Could you check a few things on this drawing? It's one solid part, dimensions in mm from its lowest x, y, z. A direction names the side the tool comes from. Give positions to 0.01 mm unless a question says otherwise; leave off trailing zeros. Order: outer loops, then holes, each group sorted by start corner. A loop starts at its lowest first (then second) coordinate and runs counter-clockwise, first axis right, second up.
Item 1: If we mould it in two halves opening along X, with no side actions, what happens to the marked faces 1, 2 and 3? For each: +X half, -X half, draft (parallel to the pull), parting line (faces both ways), or undercut.
Item 2: I want a section at D-D, the plane z = 12. Write out the boundary of the cut face in (x, y), then the cut area to 3 significant figures.
Item 3: I want a section at A-A, the plane z = 7.5. Write out the boundary of the cut face in (x, y).
Item 4: I want a section at C-C, the plane x = 7.5. Write out the boundary of the cut face in (y, z).
Item 5: Which directions (+Z, -Z, +X, -X, +Y, -Y) give clear straight access to the entire face, cutting with the end or side of a thin tool? Please do the marked faces 4, 5 and 6.
Item 6: If I drill on line 1 along Z through (x, y) = (42.5, 2); line 2 along Y through (x, z) = (25, 6.5); line 3 along X through (y, z) = (20.5, 7), over which ranges is the centre line in solid material (lowest first)?
Item 7: I'm going to push flat-ended pins straight in: pin 1 Ø5.5 at (x, y) = (25, 19) entering from +Z; pin 2 Ø7.5 at (y, z) = (21, 8.5) entering from +X; pin 3 Ø7.5 at (x, z) = (4.5, 7.5) entering from +Y; pin 4 Ø7.5 at (y, z) = (18, 9.5) entering from -X. Where does each tip first touch, or does it pass through?
Item 8: I want a section at B-B, the plane y = 19. Write out the boundary of the cut face in (x, z).
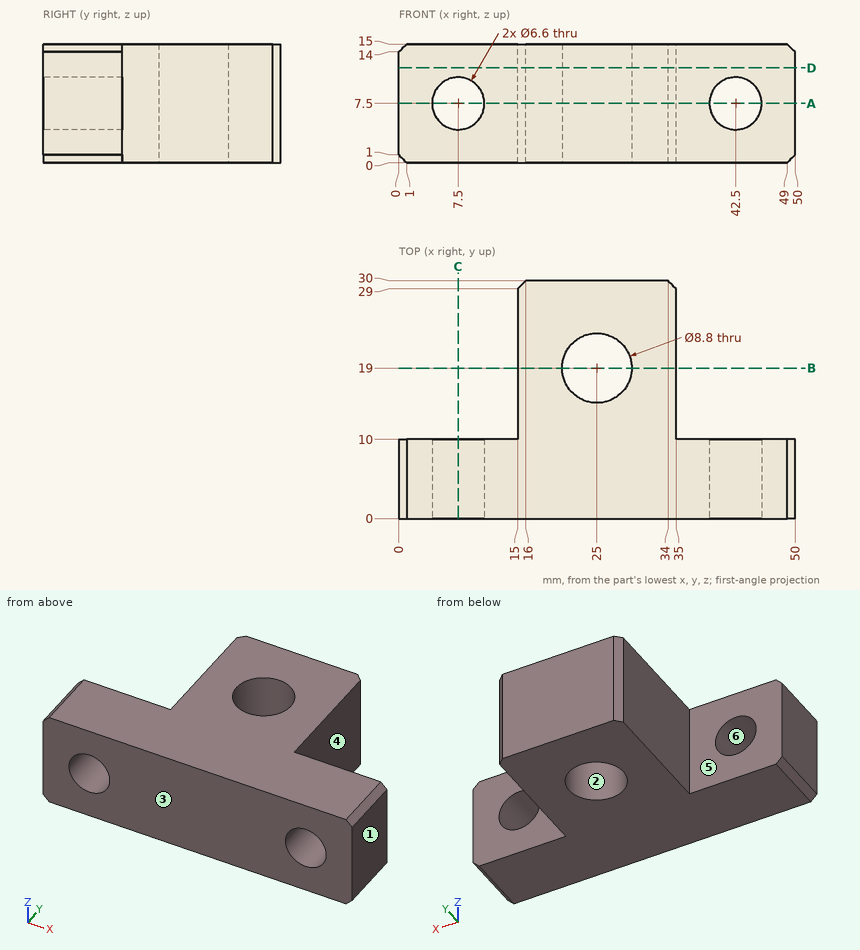
Results list:
1. face 1: +X half
1. face 2: undercut
1. face 3: draft
2. outline: (0, 0) - (50, 0) - (50, 10) - (35, 10) - (35, 29) - (34, 30) - (16, 30) - (15, 29) - (15, 10) - (0, 10) - close; hole circle Ø8.8 at (25, 19)
2. area: 838 mm2
3. outline: (0, 0) - (4.2, 0) - (4.2, 10) - (0, 10) - close; (10.8, 0) - (39.2, 0) - (39.2, 10) - (35, 10) - (35, 29) - (34, 30) - (16, 30) - (15, 29) - (15, 10) - (10.8, 10) - close; (45.8, 0) - (50, 0) - (50, 10) - (45.8, 10) - close; hole circle Ø8.8 at (25, 19)
4. outline: (0, 0) - (10, 0) - (10, 4.2) - (0, 4.2) - close; (0, 10.8) - (10, 10.8) - (10, 15) - (0, 15) - close
5. face 4: +Z, -Z, +X, +Y
5. face 5: +Z, -Z, -X, +Y
5. face 6: +Y, -Y
6. line 1: z = 0 to 4.2, 10.8 to 15
6. line 2: y = 0 to 14.6, 23.4 to 30
6. line 3: x = 15 to 20.86, 29.14 to 35
7. pin 1: passes through
7. pin 2: stops at x = 35
7. pin 3: stops at y = 10
7. pin 4: stops at x = 15
8. outline: (15, 0) - (20.6, 0) - (20.6, 15) - (15, 15) - close; (29.4, 0) - (35, 0) - (35, 15) - (29.4, 15) - close
